For this review, take the finished solid that the model builds, in its own axes (mm). A direction names the side the tool comes from. Round coordinates to 2 decimals unless told otherwise and drop trailing zeros. Loops run counter-clockwise (first coordinate to the right, second up) from the corner with the lowest first, then second, coordinate; pieces in that order, holes last.
1. Consider section A-A on z = 30.25. State the section outline as (x, y) points.
2. To check wall thickness, follow line 1 along X through (y, z) = (-24, 30); line 2 along Y through (x, z) = (6, 90.75); line 3 along Y through (x, z) = (5, 30). State the ranges of each line that lie inside material, in increasing order.
3. Tool access review of faces 5 (the flat face through (0, 2, 60)), 6 (the cylindrical face through (-31.3, -25.4, 28.6)): name each direction out of +Z, -Z, +X, -X, +Y, -Y from which nothing blocks a thin tool from reaching the whole face with its end or side.
4. Draft analysis for pull direction X (two halves, no side actions). For faces 1 (the cylindrical face through (-29.369, -25.42, 92.753)), 2 (the flat face through (5, 24.51, 60)), 3 (the flat face through (10, -3, 60)), 4 (the flat face through (-40, -26, 60)), state which applies: released by +X, released by -X, zero draft, split by the parting line, or undercut.
5. Consider section B-B on x = -30. State the section outline as (y, z) points.
6. Clearance check with flat-ended pins moving along their axes: pin 1 Ø5 at (x, z) = (-10, 90.75) entering from -Y; pin 2 Ø20 at (x, z) = (-20.5, 30.5) entering from +Y; pin 3 Ø6 at (y, z) = (-5, 62) entering from -X. State where each tip first meets the part, or that it passes through.
7. Consider section C-C on z = 62. State the section outline as (x, y) points, then the cut area to 3 significant figures.
8. Consider section D-D on y = 8.5. State the section outline as (x, z) points, then the cut area to 3 significant figures.
from build123d import *

# Parameters (mm, degrees)
EXTRUDE_1_DEPTH     = 121
CUT_EXTRUDE_2_REACH = 1320.001
SKETCH_3_R          = 2.099999998
SKETCH_3_R_2        = 2.100000002
SKETCH_5_R          = 2.1
CUT_EXTRUDE_3_DEPTH = 10


with BuildPart() as part:
    # 草图1 → 凸台-拉伸1 (new body)
    with BuildSketch(Plane.XY):
        Polygon((0, 24.51048951), (10, 24.51048951), (10, -30.48951049), (-40, -30.48951049), (-40, -20.48951049), (0, -20.48951049), align=None)
    extrude(amount=EXTRUDE_1_DEPTH)

    # 草图3 → 切除-拉伸2 (cut, up to next)
    with BuildSketch(Plane(origin=(-858.744003867, -20.48951049, -869.143932912), x_dir=(-1, 0, 0), z_dir=(0, 1, 0)), mode=Mode.PRIVATE) as cut_extrude_2_sk1:
        with Locations(Location((-848.744003867, 959.893932917, 0), (0, 0, 90))):
            Circle(SKETCH_3_R)
    cut_extrude_2_tool1 = extrude(cut_extrude_2_sk1.sketch, amount=-CUT_EXTRUDE_2_REACH, mode=Mode.PRIVATE) & part.part
    # 草图3 → 切除-拉伸2 (cut, up to next)
    with BuildSketch(Plane(origin=(-858.744003867, -20.48951049, -869.143932912), x_dir=(-1, 0, 0), z_dir=(0, 1, 0)), mode=Mode.PRIVATE) as cut_extrude_2_sk2:
        with Locations(Location((-828.744003867, 959.893932906, 0), (0, 0, 90))):
            Circle(SKETCH_3_R_2)
    cut_extrude_2_tool2 = extrude(cut_extrude_2_sk2.sketch, amount=-CUT_EXTRUDE_2_REACH, mode=Mode.PRIVATE) & part.part
    # 草图3 → 切除-拉伸2 (cut, up to next)
    with BuildSketch(Plane(origin=(-858.744003867, -20.48951049, -869.143932912), x_dir=(-1, 0, 0), z_dir=(0, 1, 0)), mode=Mode.PRIVATE) as cut_extrude_2_sk3:
        with Locations(Location((-828.744003867, 899.393932906, 0), (0, 0, 90))):
            Circle(SKETCH_3_R_2)
    cut_extrude_2_tool3 = extrude(cut_extrude_2_sk3.sketch, amount=-CUT_EXTRUDE_2_REACH, mode=Mode.PRIVATE) & part.part
    # 草图3 → 切除-拉伸2 (cut, up to next)
    with BuildSketch(Plane(origin=(-858.744003867, -20.48951049, -869.143932912), x_dir=(-1, 0, 0), z_dir=(0, 1, 0)), mode=Mode.PRIVATE) as cut_extrude_2_sk4:
        with Locations(Location((-848.744003867, 899.393932906, 0), (0, 0, 90))):
            Circle(SKETCH_3_R_2)
    cut_extrude_2_tool4 = extrude(cut_extrude_2_sk4.sketch, amount=-CUT_EXTRUDE_2_REACH, mode=Mode.PRIVATE) & part.part
    add(cut_extrude_2_tool1.solids().sort_by_distance((-10, -20.48951, 90.75))[0], mode=Mode.SUBTRACT)
    add(cut_extrude_2_tool2.solids().sort_by_distance((-30, -20.48951, 90.75))[0], mode=Mode.SUBTRACT)
    add(cut_extrude_2_tool3.solids().sort_by_distance((-30, -20.48951, 30.25))[0], mode=Mode.SUBTRACT)
    add(cut_extrude_2_tool4.solids().sort_by_distance((-10, -20.48951, 30.25))[0], mode=Mode.SUBTRACT)

    # 草图5 → 切除-拉伸3 (cut)
    with BuildSketch(Plane.ZY):
        with Locations((30.250000004, 13.26048951)):
            Circle(SKETCH_5_R)
        with Locations((30.250000004, -9.23951049)):
            Circle(SKETCH_5_R)
        with Locations((90.750000004, 13.26048951)):
            Circle(SKETCH_5_R)
        with Locations((90.750000004, -9.23951049)):
            Circle(SKETCH_5_R)
    extrude(amount=-CUT_EXTRUDE_3_DEPTH, mode=Mode.SUBTRACT)


solid = part.part
Resolved:
1. outline: (-40, -30.49) - (-32.1, -30.49) - (-32.1, -20.49) - (-40, -20.49) - close; (-27.9, -30.49) - (-12.1, -30.49) - (-12.1, -20.49) - (-27.9, -20.49) - close; (-7.9, -30.49) - (10, -30.49) - (10, -11.34) - (0, -11.34) - (0, -20.49) - (-7.9, -20.49) - close; (0, -7.14) - (10, -7.14) - (10, 11.16) - (0, 11.16) - close; (0, 15.36) - (10, 15.36) - (10, 24.51) - (0, 24.51) - close
2. line 1: x = -40 to -32.09, -27.91 to -12.09, -7.91 to 10
2. line 2: y = -30.49 to -11.34, -7.14 to 11.16, 15.36 to 24.51
2. line 3: y = -30.49 to -11.32, -7.15 to 11.18, 15.35 to 24.51
3. face 5: +Z, -Z, -X, +Y
3. face 6: +Y, -Y
4. face 1: undercut
4. face 2: zero draft
4. face 3: released by +X
4. face 4: released by -X
5. outline: (-30.49, 0) - (-20.49, 0) - (-20.49, 28.15) - (-30.49, 28.15) - close; (-30.49, 32.35) - (-20.49, 32.35) - (-20.49, 88.65) - (-30.49, 88.65) - close; (-30.49, 92.85) - (-20.49, 92.85) - (-20.49, 121) - (-30.49, 121) - close
6. pin 1: stops at y = -30.49
6. pin 2: stops at y = -20.49
6. pin 3: stops at x = 0
7. outline: (-40, -30.49) - (10, -30.49) - (10, 24.51) - (0, 24.51) - (0, -20.49) - (-40, -20.49) - close
7. area: 950 mm2
8. outline: (0, 0) - (10, 0) - (10, 121) - (0, 121) - close
8. area: 1,210 mm2
